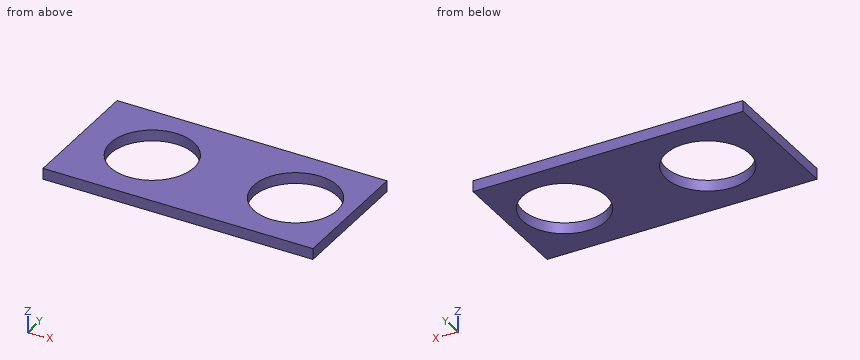
from build123d import *

# Parameters (mm, degrees)
SKETCH1_W           = 245
SKETCH1_H           = 118
SKETCH1_R           = 38
BOSS_EXTRUDE1_DEPTH = 10


with BuildPart() as part:
    # Sketch1 → Boss-Extrude1 (new body)
    with BuildSketch(Plane.XY):
        with Locations((122.5, 59)):
            Rectangle(SKETCH1_W, SKETCH1_H)
        with Locations((195, 60)):
            Circle(SKETCH1_R, mode=Mode.SUBTRACT)
        with Locations((65, 60)):
            Circle(SKETCH1_R, mode=Mode.SUBTRACT)
    extrude(amount=BOSS_EXTRUDE1_DEPTH)


solid = part.part
CAD build for the part. Positions are in the model's coordinates, mm. Round coordinates to 2 decimals unless told otherwise and drop trailing zeros. Loops run counter-clockwise (first coordinate to the right, second up) from the corner with the lowest first, then second, coordinate; pieces in that order, holes last.
(1) Wall check: line 1 along Y through (x, z) = (65, 5.25); line 2 along X through (y, z) = (95, 4.5); line 3 along X through (y, z) = (52.5, 9). Give the ranges that are in metal, low to high.
(2) Cut at C-C (z = 3.5). Give the cut face in (x, y).
(3) Cut at D-D (y = 89.5). Give the cut face in (x, z).
(4) Cut at A-A (y = 60). Give the cut face in (x, z), plus the area to 3 significant figures.
(5) Cut at B-B (x = 65). Give the cut face in (y, z), plus the area to 3 significant figures.
Findings below:
1. line 1: y = 0 to 22, 98 to 118
1. line 2: x = 0 to 50.2, 79.8 to 180.2, 209.8 to 245
1. line 3: x = 0 to 27.75, 102.25 to 157.75, 232.25 to 245
2. outline: (0, 0) - (245, 0) - (245, 118) - (0, 118) - close; hole circle Ø76 at (65, 60); hole circle Ø76 at (195, 60)
3. outline: (0, 0) - (41.05, 0) - (41.05, 10) - (0, 10) - close; (88.95, 0) - (171.05, 0) - (171.05, 10) - (88.95, 10) - close; (218.95, 0) - (245, 0) - (245, 10) - (218.95, 10) - close
4. outline: (0, 0) - (27, 0) - (27, 10) - (0, 10) - close; (103, 0) - (157, 0) - (157, 10) - (103, 10) - close; (233, 0) - (245, 0) - (245, 10) - (233, 10) - close
4. area: 930 mm2
5. outline: (0, 0) - (22, 0) - (22, 10) - (0, 10) - close; (98, 0) - (118, 0) - (118, 10) - (98, 10) - close
5. area: 420 mm2
